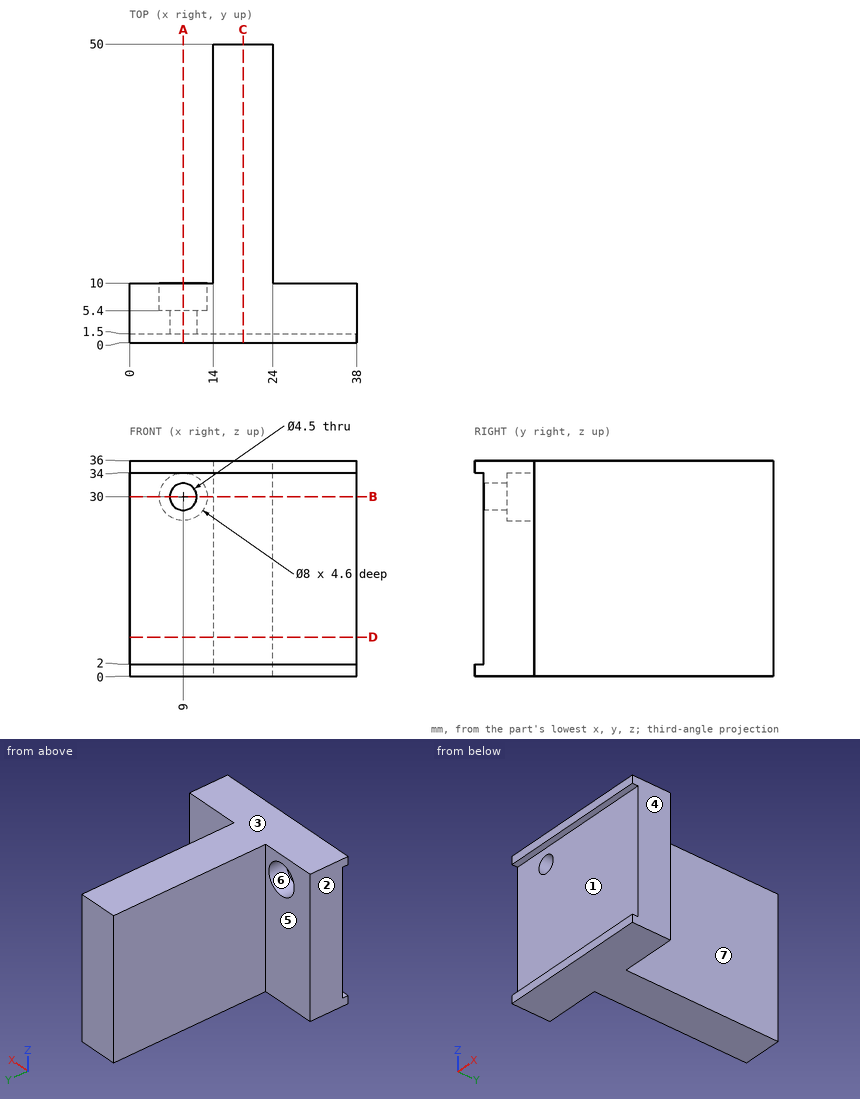
Can you work these out from the drawing? Everything is in mm from the part's minimum corner. A direction names the side the tool comes from. Round coordinates to 2 decimals unless told otherwise and drop trailing zeros. Write each loop counter-clockwise with the first axis right and the second up, starting at its lowest first coordinate (ties: lowest second). Pieces come first, ordered by that corner, then holes. Notation, with made-up numbers: (57, 28) - (95, 28) arc R18 ccw to (95, 48) - close; hole circle Ø10 at (5.25, -29.5). An arc over 180 degrees is marked (long way). Write each question's results on one line, items separated by ' | '. Start each with the question number.
1) Please list where these lines run through material, in increasing order: line 1 (X direction, y = 6.5, z = 30); line 2 (X direction, y = 3.9, z = 30); line 3 (Y direction, x = 20.5, z = 8.5).
2) Suppose I cut it at C-C (x = 19). List the corners of the cut face in (y, z) for me, and give its area (3 significant figures).
3) Suppose I cut it at D-D (z = 6.5). List the corners of the cut face in (x, y) for me, and give its area (3 significant figures).
4) Which directions (+Z, -Z, +X, -X, +Y, -Y) give clear straight access to the entire face, cutting with the end or side of a thin tool? Please do the marked faces 4, 5, 6 and 7.
5) Suppose I cut it at A-A (x = 9). List the corners of the cut face in (y, z) for me.
6) For pin 1 Ø1.5 at (y, z) = (32, 31.5) entering from +X; pin 2 Ø15.5 at (x, z) = (6, 11.5) entering from +Y; pin 3 Ø9.5 at (x, z) = (19, 25.5) entering from -Y, each with a flat end and sliding along its axis, tell me the tip position at first contact or that it passes through.
7) Suppose I cut it at B-B (z = 30). List the corners of the cut face in (x, y) for me, and give its area (3 significant figures).
8) We'd pull the mould along Z, two halves only. Please class the marked faces 1, 2 and 3: released by +Z, released by -Z, zero draft, split by the parting line, or undercut.
Here are the results:
1) line 1: x = 0 to 5, 13 to 38 | line 2: x = 0 to 6.75, 11.25 to 38 | line 3: y = 1.5 to 50
2) outline: (0, 0) - (50, 0) - (50, 36) - (0, 36) - (0, 34) - (1.5, 34) - (1.5, 2) - (0, 2) - close | area: 1,750 mm2
3) outline: (0, 1.5) - (38, 1.5) - (38, 10) - (24, 10) - (24, 50) - (14, 50) - (14, 10) - (0, 10) - close | area: 723 mm2
4) face 4: +Z, -Z, +X, +Y, -Y | face 5: +Z, -Z, -X, +Y | face 6: +Y | face 7: +Z, -Z, +X, +Y
5) outline: (0, 0) - (10, 0) - (10, 26) - (5.4, 26) - (5.4, 27.75) - (1.5, 27.75) - (1.5, 2) - (0, 2) - close; (0, 34) - (1.5, 34) - (1.5, 32.25) - (5.4, 32.25) - (5.4, 34) - (10, 34) - (10, 36) - (0, 36) - close
6) pin 1: stops at x = 24 | pin 2: stops at y = 10 | pin 3: stops at y = 1.5
7) outline: (0, 1.5) - (6.75, 1.5) - (6.75, 5.4) - (5, 5.4) - (5, 10) - (0, 10) - close; (11.25, 1.5) - (38, 1.5) - (38, 10) - (24, 10) - (24, 50) - (14, 50) - (14, 10) - (13, 10) - (13, 5.4) - (11.25, 5.4) - close | area: 669 mm2
8) face 1: undercut | face 2: zero draft | face 3: released by +Z
